Input: part model. Units: mm. Frame: model coordinates. A direction names the side the tool comes from. Coordinates: 2 decimals unless noted, no trailing zeros. Loops run counter-clockwise (first coordinate to the right, second up) from the corner with the lowest first, then second, coordinate; pieces in that order, holes last. Notation, with made-up numbers: (-35, -21.5) -> (-27, -21.5) arc R26 cw to (-27, 10.5) -> close; hole circle Ø6 at (23.5, 62). An arc over 180 degrees is marked (long way). Answer as a JSON object with one key per item and string values.
from build123d import *

# Parameters (mm, degrees)
SKETCH1_W           = 50
SKETCH1_H           = 50
BOSS_EXTRUDE1_DEPTH = 100
SKETCH4_W           = 30
SKETCH4_H           = 50
CUT_EXTRUDE2_DEPTH  = 35
SKETCH6_R           = 16
CUT_EXTRUDE3_DEPTH  = 10
SKETCH8_R           = 4
CUT_EXTRUDE6_DEPTH  = 10
CUT_EXTRUDE7_START  = -10
SKETCH9_R           = 4
CUT_EXTRUDE7_DEPTH  = 10


with BuildPart() as part:
    # Sketch1 → Boss-Extrude1 (new body)
    with BuildSketch(Plane(origin=(0, 0, 0), x_dir=(1, 0, 0), z_dir=(0, 1, 0))):
        Rectangle(SKETCH1_W, SKETCH1_H)
    extrude(amount=BOSS_EXTRUDE1_DEPTH)

    # Sketch4 → Cut-Extrude2 (cut)
    with BuildSketch(Plane.XZ):
        Rectangle(SKETCH4_W, SKETCH4_H)
    extrude(amount=-CUT_EXTRUDE2_DEPTH, mode=Mode.SUBTRACT)

    # Sketch6 → Cut-Extrude3 (cut)
    with BuildSketch(Plane(origin=(0, 100, 0), x_dir=(1, 0, 0), z_dir=(0, 1, 0))):
        with Locations(Location((0, 0, 0), (0, 0, 270))):
            Circle(SKETCH6_R)
    extrude(amount=-CUT_EXTRUDE3_DEPTH, mode=Mode.SUBTRACT)

    # Sketch8 → Cut-Extrude6 (cut)
    with BuildSketch(Plane.ZY.offset(25)):
        with Locations((-16, 80)):
            Circle(SKETCH8_R)
        with Locations((16, 80)):
            Circle(SKETCH8_R)
        with Locations((16, 50)):
            Circle(SKETCH8_R)
        with Locations((-16, 50)):
            Circle(SKETCH8_R)
    extrude(amount=-CUT_EXTRUDE6_DEPTH, mode=Mode.SUBTRACT)

    # Sketch9 → Cut-Extrude7 (cut)
    with BuildSketch(Plane(origin=(25, 0, 0), x_dir=(0, 0, -1), z_dir=(1, 0, 0)).offset(CUT_EXTRUDE7_START)):
        with Locations(Location((-16, 80, 0), (0, 0, 180))):
            Circle(SKETCH9_R)
        with Locations(Location((-16, 50, 0), (0, 0, 180))):
            Circle(SKETCH9_R)
        with Locations(Location((16, 50, 0), (0, 0, 180))):
            Circle(SKETCH9_R)
        with Locations(Location((16, 80, 0), (0, 0, 180))):
            Circle(SKETCH9_R)
    extrude(amount=CUT_EXTRUDE7_DEPTH, mode=Mode.SUBTRACT)


solid = part.part
1. Pin query (flat end, axial travel): P1, Ø4, axis at y = 81.5, z = -15.5, coming from the -X side; P2, Ø13, axis at y = 50, z = 16, coming from the +X side; P3, Ø9.5, axis at x = 2, z = -8, coming from the +Y side; P4, Ø5, axis at y = 80, z = 16, coming from the +X side. Return the tip coordinate at first contact, or that it passes through.
Reply:
{"P1": "stops at x = -15", "P2": "stops at x = 25", "P3": "stops at y = 90", "P4": "stops at x = 15"}
2. Section query B-B (x = 0). Return loops of the section in (y, z).
Reply:
{"outline": "(35, -25) -> (100, -25) -> (100, -16) -> (90, -16) -> (90, 16) -> (100, 16) -> (100, 25) -> (35, 25) -> close"}
3. Access query for faces 4 (the face through (-20, 0, 0)), 5 (the face through (19.9, 52.4, -19.2)), 6 (the face through (-20.07, 76.095, -16.867)), 7 (the face through (-15.62, 95.07, -3.47)), 8 (the face through (-15, 17, 0)). Directions: +Z, -Z, +X, -X, +Y, -Y. A direction counts if a zero-diameter tool reaches every point of the face in a straight line with its end or side. Return the directions, or none.
Reply:
{"face 4": "+Z, -Z, +X, -X, -Y", "face 5": "+X", "face 6": "-X", "face 7": "+Y", "face 8": "+Z, -Z, -Y"}
4. Line query: line 1 along Y through (x, z) = (17.5, 16); line 2 along Z through (x, y) = (21, 50); line 3 along X through (y, z) = (34, -2.5). Output: solid intervals per line, ascending.
Reply:
{"line 1": "y = 0 to 46, 54 to 76, 84 to 100", "line 2": "z = -25 to -20, -12 to 12, 20 to 25", "line 3": "x = -25 to -15, 15 to 25"}
5. Section query C-C (z = 10). Return loops of the section in (x, y).
Reply:
{"outline": "(-25, 0) -> (-15, 0) -> (-15, 35) -> (15, 35) -> (15, 0) -> (25, 0) -> (25, 100) -> (12.49, 100) -> (12.49, 90) -> (-12.49, 90) -> (-12.49, 100) -> (-25, 100) -> close"}
6. Section query D-D (y = 80). Return loops of the section in (x, z), plus the area to 3 significant figures.
Reply:
{"outline": "(-25, -25) -> (25, -25) -> (25, -20) -> (15, -20) -> (15, -12) -> (25, -12) -> (25, 12) -> (15, 12) -> (15, 20) -> (25, 20) -> (25, 25) -> (-25, 25) -> (-25, 20) -> (-15, 20) -> (-15, 12) -> (-25, 12) -> (-25, -12) -> (-15, -12) -> (-15, -20) -> (-25, -20) -> close", "area": "2,180 mm2"}
7. Section query A-A (y = 7). Return loops of the section in (x, z), plus the area to 3 significant figures.
Reply:
{"outline": "(-25, -25) -> (-15, -25) -> (-15, 25) -> (-25, 25) -> close; (15, -25) -> (25, -25) -> (25, 25) -> (15, 25) -> close", "area": "1,000 mm2"}
8. Mould query, pull axis Y, two halves, no side actions, for faces 1 (the face through (15, 50, 16)), 2 (the face through (20, 0, 0)), 3 (the face through (25, 49, 0)). Classes: pulls with the +Y half, pulls with the -Y half, needs draft (parallel to the pull), parting line crosses it, or undercut.
Reply:
{"face 1": "undercut", "face 2": "pulls with the -Y half", "face 3": "needs draft"}
